Work out the finished part from the listing and answer in its coordinate system (mm). A direction names the side the tool comes from. Round coordinates to 2 decimals unless told otherwise and drop trailing zeros. Loops run counter-clockwise (first coordinate to the right, second up) from the corner with the lowest first, then second, coordinate; pieces in that order, holes last. Notation, with made-up numbers: M 23.25,80 L 74.25,80 A9 ccw 74.25,87 Z; hole C -2.5,39 d2. An arc over 180 degrees is marked long. One line per item, written item: value.
```python
from build123d import *

# Parameters (mm, degrees)
SKETCH_1_W                = 140
SKETCH_1_H                = 36
EXTRUDE_1_DEPTH           = 25
HOLE_WIZARD_1_D           = 6.6
HOLE_WIZARD_1_CBORE_D     = 11
HOLE_WIZARD_1_CBORE_DEPTH = 7
CHAMFER_1_SIZE            = 2


with BuildPart() as part:
    # 草图1 → 凸台-拉伸1 (new body)
    with BuildSketch(Plane(origin=(0, 0, 0), x_dir=(1, 0, 0), z_dir=(0, 1, 0))):
        with Locations((70, 18)):
            Rectangle(SKETCH_1_W, SKETCH_1_H)
    extrude(amount=EXTRUDE_1_DEPTH)

    # 打孔尺寸(%根据)内六角圆柱头螺钉的类型1 (through all)
    with Locations(Plane(origin=(0, 25, 0), x_dir=(1, 0, 0), z_dir=(0, 1, 0))):
        with Locations((32.5, 18), (107.5, 18)):
            CounterBoreHole(HOLE_WIZARD_1_D / 2, HOLE_WIZARD_1_CBORE_D / 2, HOLE_WIZARD_1_CBORE_DEPTH)

    # 倒角1
    chamfer_1_edges = [part.edges().sort_by_distance(p)[0] for p in [
        (0, 12.5, -36),
        (140, 12.5, -36),
        (140, 12.5, 0),
        (0, 12.5, 0),
    ]]
    chamfer(chamfer_1_edges, length=CHAMFER_1_SIZE)


solid = part.part
```
1) Find the intervals of material crossed by probe 1 along X at (y, z) = (10.75, -18); probe 2 along X at (y, z) = (23.75, -18); probe 3 along Z at (x, y) = (107.5, 12.75), in increasing order. Write a range as from..to.
Check values:
probe 1: 0..29.2, 35.8..104.2, 110.8..140
probe 2: 0..27, 38..102, 113..140
probe 3: -36..-21.3, -14.7..0
2) This flat-tipped pin is pushed along its axis until it touches: pin 1 (12 mm diameter, centred on x = 34, z = -17.5, fed in from +Y). Where does it stop, or does it pass through?
Check values:
pin 1: y = 25
3) Find section C-C (x = 32.5). Give the vertices of the cut face in (y, z), then the cut area to 3 significant figures.
Check values:
outline: M 0,-36 L 25,-36 L 25,-23.5 L 18,-23.5 L 18,-21.3 L 0,-21.3 Z; M 0,-14.7 L 18,-14.7 L 18,-12.5 L 25,-12.5 L 25,0 L 0,0 Z
area: 704 mm2
4) The mould has two halves that part along X. Classify faces 1 (the face through (69, 0, -18)), 2 (the face through (140, 12, -18)), 3 (the face through (36, 18, -18)): +X half, -X half, draft (parallel to the pull), parting line (faces both ways), or undercut.
Check values:
face 1: draft
face 2: +X half
face 3: undercut
5) Find section A-A (z = -18). Give the vertices of the cut face in (x, y).
Check values:
outline: M 0,0 L 29.2,0 L 29.2,18 L 27,18 L 27,25 L 0,25 Z; M 35.8,0 L 104.2,0 L 104.2,18 L 102,18 L 102,25 L 38,25 L 38,18 L 35.8,18 Z; M 110.8,0 L 140,0 L 140,25 L 113,25 L 113,18 L 110.8,18 Z
6) For faces 4 (the face through (27, 22, -18)), 5 (the face through (69, 12, -36)), determine the directions among +Z, -Z, +X, -X, +Y, -Y from which every point of the face is accessible in a straight line to the end or side of a thin tool.
Check values:
face 4: +Y
face 5: -Z, +X, -X, +Y, -Y
7) Find section B-B (y = 11.5). Give the vertices of the cut face in (x, z).
Check values:
outline: M 0,-34 L 2,-36 L 138,-36 L 140,-34 L 140,-2 L 138,0 L 2,0 L 0,-2 Z; hole C 32.5,-18 d6.6; hole C 107.5,-18 d6.6
8) Find section D-D (y = 23.5). Give the vertices of the cut face in (x, z).
Check values:
outline: M 0,-34 L 2,-36 L 138,-36 L 140,-34 L 140,-2 L 138,0 L 2,0 L 0,-2 Z; hole C 32.5,-18 d11; hole C 107.5,-18 d11
